Can you work these out from the drawing? Everything is in mm from the part's minimum corner. A direction names the side the tool comes from. Round coordinates to 2 decimals unless told otherwise and drop trailing zeros. Loops run counter-clockwise (first coordinate to the right, second up) from the corner with the lowest first, then second, coordinate; pieces in that order, holes last. Notation, with made-up numbers: (26, 34.25) -> (55, 34.25) arc R8 ccw to (55, 38.25) -> close; hole circle Ø3 at (54.25, 12.5). An arc over 180 degrees is marked (long way). Answer as a JSON object with one key per item and string values.
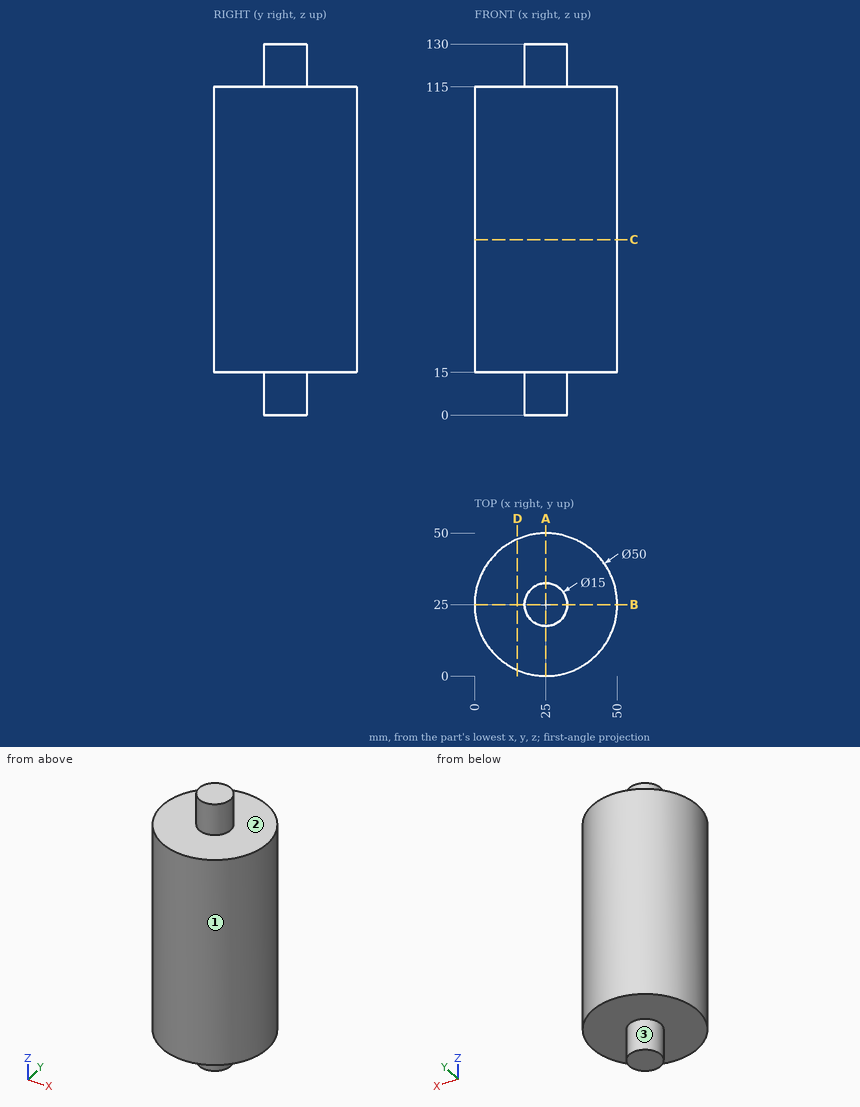
Q1. I want a section at C-C, the plane z = 61.5. Write out the boundary of the cut face in (x, y).
Determined:
{"outline": "circle Ø50 at (25, 25)"}
Q2. I want a section at A-A, the plane x = 25. Write out the boundary of the cut face in (y, z).
Determined:
{"outline": "(0, 15) -> (17.5, 15) -> (17.5, 0) -> (32.5, 0) -> (32.5, 15) -> (50, 15) -> (50, 115) -> (32.5, 115) -> (32.5, 130) -> (17.5, 130) -> (17.5, 115) -> (0, 115) -> close"}
Q3. I want a section at D-D, the plane x = 15. Write out the boundary of the cut face in (y, z).
Determined:
{"outline": "(2.09, 15) -> (47.91, 15) -> (47.91, 115) -> (2.09, 115) -> close"}
Q4. I'm going to push flat-ended pins straight in: pin 1 (2 mm diameter, centred on x = 12, z = 83.5, fed in from +Y); pin 2 (12 mm diameter, centred on x = 23, z = 51, fed in from +Y); pin 3 (1.5 mm diameter, centred on x = 12, z = 42, fed in from -Y). Where does each tip first touch, or does it pass through?
Determined:
{"pin 1": "y = 46.93", "pin 2": "y = 50", "pin 3": "y = 3.21"}
Q5. If I drill on L1, parallel to Z at x = 41.5, y = 23; L2, parallel to X at y = 28, z = 66; L3, parallel to Y at x = 25.5, z = 48 (3 decimals), over which ranges is the centre line in solid material (lowest first)? Write a range as [from, to].
Determined:
{"L1": "[15, 115]", "L2": "[0.18, 49.82]", "L3": "[0.005, 49.995]"}
Q6. On a 3-axis mill with a long thin cutter (end or side, diameter ignored), from which of +Z, -Z, +X, -X, +Y, -Y can I reach the whole of each face in a straight line? I mean the marked faces 1, 2 and 3. Say none if no direction works.
Determined:
{"face 1": "+Z, -Z", "face 2": "+Z", "face 3": "-Z"}
